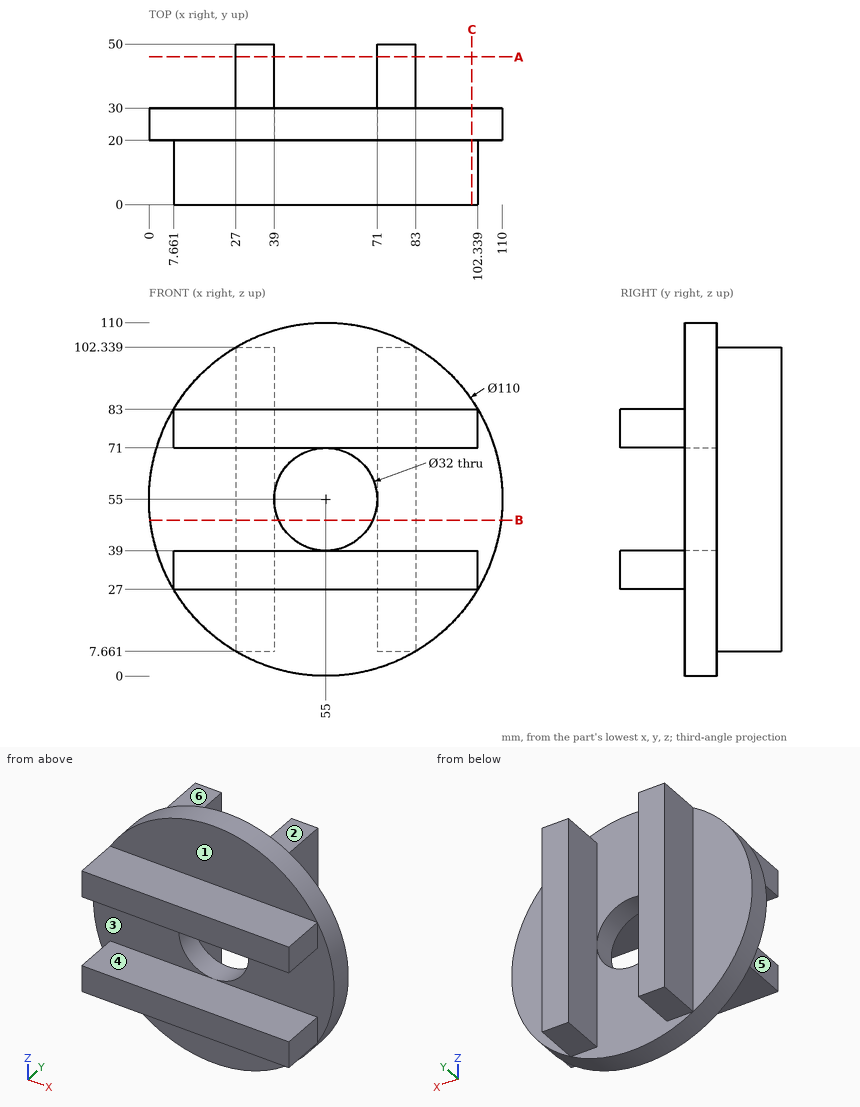
Design review of the part shown in the three views and the two pictorial views. Dimensions are in mm from the part's minimum x, y and z. A direction names the side the tool comes from. Give positions to 0.01 mm unless a question says otherwise; leave off trailing zeros. Loops run counter-clockwise (first coordinate to the right, second up) from the corner with the lowest first, then second, coordinate; pieces in that order, holes last. Notation, with made-up numbers: M 11.25,68.5 L 27.25,68.5 A9 ccw 27.25,81.5 Z; hole C 73.5,31.5 d9. An arc over 180 degrees is marked long. Answer as a JSON object with one key per item and string values. Group by question number.
Q1. For probe 1 along X at (y, z) = (23.5, 55); probe 2 along X at (y, z) = (40.5, 85.5), list the stretches that pass through material, from the lowest coordinate up. Write a range as [from, to].
Q2. Add section C-C on x = 100.5. Give the boundary of the cut face in (y, z).
Q3. Tool access review of the marked faces 4, 5 and 6: name each direction out of +Z, -Z, +X, -X, +Y, -Y from which nothing blocks a thin tool from reaching the whole face with its end or side.
Q4. Insertion check: P1, Ø6, axis at x = 27, y = 10.5, coming from the +Z side; P2, Ø10, axis at y = 44, z = 95.5, coming from the -X side; P3, Ø22, axis at x = 63.5, y = 13, coming from the +Z side; P4, Ø16.5, axis at x = 68, z = 38, coming from the +Y side. Each pin has a flat end and moves straight along its axis. Give the tip position at first contact, or say it passes through.
Q5. Add section B-B on z = 48.5. Give the boundary of the cut face in (x, y), and give its area (3 significant figures).
Q6. Mouldability with a two-part tool opening along Z and no side actions: class the marked faces 1, 2 and 3 as +Z half, -Z half, draft (parallel to the pull), parting line (faces both ways), or undercut.
Q7. Add section A-A on y = 46. Give the boundary of the cut face in (x, z), and give its area (3 significant figures).
Checked values:
{
 "1": {"probe 1": "[0, 39], [71, 110]", "probe 2": "[27, 39], [71, 83]"},
 "2": {"outline": "M 0,27 L 20,27 L 20,24.1 L 30,24.1 L 30,85.9 L 20,85.9 L 20,83 L 0,83 L 0,71 L 20,71 L 20,39 L 0,39 Z"},
 "3": {"face 4": "+X, -X, -Y", "face 5": "+Z, -Z, -X, -Y", "face 6": "+Z, +X, -X, +Y"},
 "4": {"P1": "z = 83", "P2": "x = 27", "P3": "z = 110", "P4": "y = 50"},
 "5": {"outline": "M 0.39,20 L 40.38,20 L 40.38,30 L 39,30 L 39,50 L 27,50 L 27,30 L 0.39,30 Z; M 69.62,20 L 109.61,20 L 109.61,30 L 83,30 L 83,50 L 71,50 L 71,30 L 69.62,30 Z", "area": "1,280 mm²"},
 "6": {"face 1": "draft", "face 2": "+Z half", "face 3": "undercut"},
 "7": {"outline": "M 27,7.66 L 39,7.66 L 39,102.34 L 27,102.34 Z; M 71,7.66 L 83,7.66 L 83,102.34 L 71,102.34 Z", "area": "2,270 mm²"}
}
